```python
from build123d import *

# Parameters (mm, degrees)
SKETCH_1_W          = 35
SKETCH_1_H          = 12
EXTRUDE_1_DEPTH     = 207.5
SKETCH_2_R          = 10.5
SKETCH_2_R_2        = 5.5
CUT_EXTRUDE_1_DEPTH = 12


with BuildPart() as part:
    # 草图1 → 凸台-拉伸1 (new, symmetric)
    with BuildSketch(Plane.XY):
        Rectangle(SKETCH_1_W, SKETCH_1_H)
    extrude(amount=EXTRUDE_1_DEPTH, both=True)

    # 草图2 → 切除-拉伸1 (cut)
    with BuildSketch(Plane(origin=(0, 6, 0), x_dir=(1, 0, 0), z_dir=(0, 1, 0))):
        with Locations(Location((0, 187.5, 0), (0, 0, 270))):
            Circle(SKETCH_2_R)
        with Locations(Location((0, -152.5, 0), (0, 0, 270))):
            Circle(SKETCH_2_R_2)
        with Locations(Location((0, -172.5, 0), (0, 0, 270))):
            Circle(SKETCH_2_R_2)
    extrude(amount=-CUT_EXTRUDE_1_DEPTH, mode=Mode.SUBTRACT)


solid = part.part
```
Verification items for the finished model (mm, model axes). Give positions to 0.01 mm unless a question says otherwise; leave off trailing zeros. Order: outer loops, then holes, each group sorted by start corner. A loop starts at its lowest first (then second) coordinate and runs counter-clockwise, first axis right, second up. Notation, with made-up numbers: (-29.5, 10.25) -> (8.5, 10.25) arc R26 cw to (8.5, 44.25) -> close; hole circle Ø8 at (33, 69). An arc over 180 degrees is marked (long way). Use a Markdown table: item, result.
1) Section check A-A, the plane x = 0. Record the boundary of the cut face in (y, z).
Results:
| item | result |
|---|---|
| outline | (-6, -207.5) -> (6, -207.5) -> (6, -198) -> (-6, -198) -> close; (-6, -177) -> (6, -177) -> (6, 147) -> (-6, 147) -> close; (-6, 158) -> (6, 158) -> (6, 167) -> (-6, 167) -> close; (-6, 178) -> (6, 178) -> (6, 207.5) -> (-6, 207.5) -> close |
2) Material ranges on probe 1 along X at (y, z) = (1.25, -187.5); probe 2 along X at (y, z) = (-1, 152.5); probe 3 along Z at (x, y) = (-4, 3), recorded low to high.
Results:
| item | result |
|---|---|
| probe 1 | -17.5 to -10.5, 10.5 to 17.5 |
| probe 2 | -17.5 to -5.5, 5.5 to 17.5 |
| probe 3 | -207.5 to -197.21, -177.79 to 148.73, 156.27 to 168.73, 176.27 to 207.5 |
3) Section check B-B, the plane z = -187.5. Record the boundary of the cut face in (x, y).
Results:
| item | result |
|---|---|
| outline | (-17.5, -6) -> (-10.5, -6) -> (-10.5, 6) -> (-17.5, 6) -> close; (10.5, -6) -> (17.5, -6) -> (17.5, 6) -> (10.5, 6) -> close |
4) Section check D-D, the plane z = 172.5. Record the boundary of the cut face in (x, y).
Results:
| item | result |
|---|---|
| outline | (-17.5, -6) -> (-5.5, -6) -> (-5.5, 6) -> (-17.5, 6) -> close; (5.5, -6) -> (17.5, -6) -> (17.5, 6) -> (5.5, 6) -> close |
5) Mould release check, pull along X, two halves, no side actions. Record for faces 1 (the flat face through (17.5, 0, 3)), 2 (the flat face through (0, 0, -207.5)), 3 (the flat face through (-17.5, 0, 3)), 4 (the cylindrical face through (0, 0, 167)): pulls with the +X half, pulls with the -X half, needs draft (parallel to the pull), parting line crosses it, or undercut.
Results:
| item | result |
|---|---|
| face 1 | pulls with the +X half |
| face 2 | needs draft |
| face 3 | pulls with the -X half |
| face 4 | undercut |
6) Depth check by flat-ended pin: pin 1 Ø9 at (x, z) = (0, 172.5) entering from +Y; pin 2 Ø14.5 at (x, z) = (0, 152.5) entering from +Y. Enter the tip coordinate at first touch or a pass-through.
Results:
| item | result |
|---|---|
| pin 1 | through |
| pin 2 | y = 6 |
7) Section check C-C, the plane y = -1.25. Record the boundary of the cut face in (x, z).
Results:
| item | result |
|---|---|
| outline | (-17.5, -207.5) -> (17.5, -207.5) -> (17.5, 207.5) -> (-17.5, 207.5) -> close; hole circle Ø21 at (0, -187.5); hole circle Ø11 at (0, 152.5); hole circle Ø11 at (0, 172.5) |
